from build123d import *

# Parameters (mm, degrees)
SKETCH_1_W      = 8
SKETCH_1_H      = 16.45
SKETCH_1_R      = 1.25
EXTRUDE_1_DEPTH = 3
FILLET_1_R      = 1


with BuildPart() as part:
    # 草图1 → 凸台-拉伸1 (new body)
    with BuildSketch(Plane.XY):
        with Locations((0, 4.825)):
            Rectangle(SKETCH_1_W, SKETCH_1_H)
        Circle(SKETCH_1_R, mode=Mode.SUBTRACT)
        with Locations((0, 8.25)):
            Circle(SKETCH_1_R, mode=Mode.SUBTRACT)
    extrude(amount=EXTRUDE_1_DEPTH)

    # 圆角1
    fillet_1_edges = [part.edges().sort_by_distance(p)[0] for p in [
        (4, -3.4, 1.5),
        (-4, -3.4, 1.5),
        (-4, 13.05, 1.5),
        (4, 13.05, 1.5),
    ]]
    fillet(fillet_1_edges, radius=FILLET_1_R)


solid = part.part
Part model, mm, in its own coordinate system. Coordinates: 2 decimals unless noted, no trailing zeros. Order: outer loops, then holes, each group sorted by start corner. A loop starts at its lowest first (then second) coordinate and runs counter-clockwise, first axis right, second up. Notation, with made-up numbers: M 81,31.25 L 118,31.25 A24 cw 118,53.25 Z; hole C 86.25,81 d10. An arc over 180 degrees is marked long. Use a Markdown table: item, result.
(1) Cut at C-C on z = 0.95. Write the cut outline in (x, y), then the cut area to 3 significant figures.
A:
| item | result |
|---|---|
| outline | M -4,-2.4 A1 ccw -3,-3.4 L 3,-3.4 A1 ccw 4,-2.4 L 4,12.05 A1 ccw 3,13.05 L -3,13.05 A1 ccw -4,12.05 Z; hole C 0,0 d2.5; hole C 0,8.25 d2.5 |
| area | 121 mm^2 |
(2) Cut at B-B on x = -1. Write the cut outline in (y, z).
A:
| item | result |
|---|---|
| outline | M -3.4,0 L -0.75,0 L -0.75,3 L -3.4,3 Z; M 0.75,0 L 7.5,0 L 7.5,3 L 0.75,3 Z; M 9,0 L 13.05,0 L 13.05,3 L 9,3 Z |
(3) Probe L1, parallel to Y at x = 0, z = 2; L2, parallel to Y at x = 0.5, z = 2; L3, parallel to X at y = 8.5, z = 0.7. List the from-to ranges inside material, lowest first.
A:
| item | result |
|---|---|
| L1 | y = -3.4 to -1.25, 1.25 to 7, 9.5 to 13.05 |
| L2 | y = -3.4 to -1.15, 1.15 to 7.1, 9.4 to 13.05 |
| L3 | x = -4 to -1.22, 1.22 to 4 |
(4) Pull direction X, two halves, no side cores. Call faces 1 (the cylindrical face through (1, 9, 1)), 2 (the flat face through (0, -3.4, 1)), 3 (the cylindrical face through (3.699, 12.765, 1.521)), 4 (the cylindrical face through (-0.27, -1.22, 1.48)): released by +X, released by -X, zero draft, split by the parting line, or undercut.
A:
| item | result |
|---|---|
| face 1 | undercut |
| face 2 | zero draft |
| face 3 | released by +X |
| face 4 | undercut |
(5) Cut at D-D on x = 0. Write the cut outline in (y, z).
A:
| item | result |
|---|---|
| outline | M -3.4,0 L -1.25,0 L -1.25,3 L -3.4,3 Z; M 1.25,0 L 7,0 L 7,3 L 1.25,3 Z; M 9.5,0 L 13.05,0 L 13.05,3 L 9.5,3 Z |
(6) Cut at A-A on y = 0. Write the cut outline in (x, z), then the cut area to 3 significant figures.
A:
| item | result |
|---|---|
| outline | M -4,0 L -1.25,0 L -1.25,3 L -4,3 Z; M 1.25,0 L 4,0 L 4,3 L 1.25,3 Z |
| area | 16.5 mm^2 |
